Input: dimensioned drawing with shaded views. Units: mm. Origin: part minimum x, y, z. A direction names the side the tool comes from. Coordinates: 2 decimals unless noted, no trailing zeros. Loops run counter-clockwise (first coordinate to the right, second up) from the corner with the lowest first, then second, coordinate; pieces in that order, holes last.
Item 1: Pin query (flat end, axial travel): pin 1 Ø13 at (x, y) = (29, 46.5) entering from -Z; pin 2 Ø12 at (y, z) = (37.5, 120.5) entering from +X. Return the tip coordinate at first contact, or that it passes through.
Item 2: Section query C-C, the plane z = 124. Return the cut outline in (x, y), then the cut area to 3 significant figures.
Item 3: Line query: probe 1 along X at (y, z) = (3, 76.5); probe 2 along Z at (x, y) = (9.5, 31). Output: solid intervals per line, ascending.
Item 4: Section query B-B, the plane x = 30. Return the cut outline in (y, z), then the cut area to 3 significant figures.
Item 5: Reachability of the marked faces 1, 2 and 3 from +Z, -Z, +X, -X, +Y, -Y: full face, straight path, thin tool, end or side. Return the list, or none.
Item 6: Section query A-A, the plane y = 31. Return the cut outline in (x, z), then the cut area to 3 significant figures.
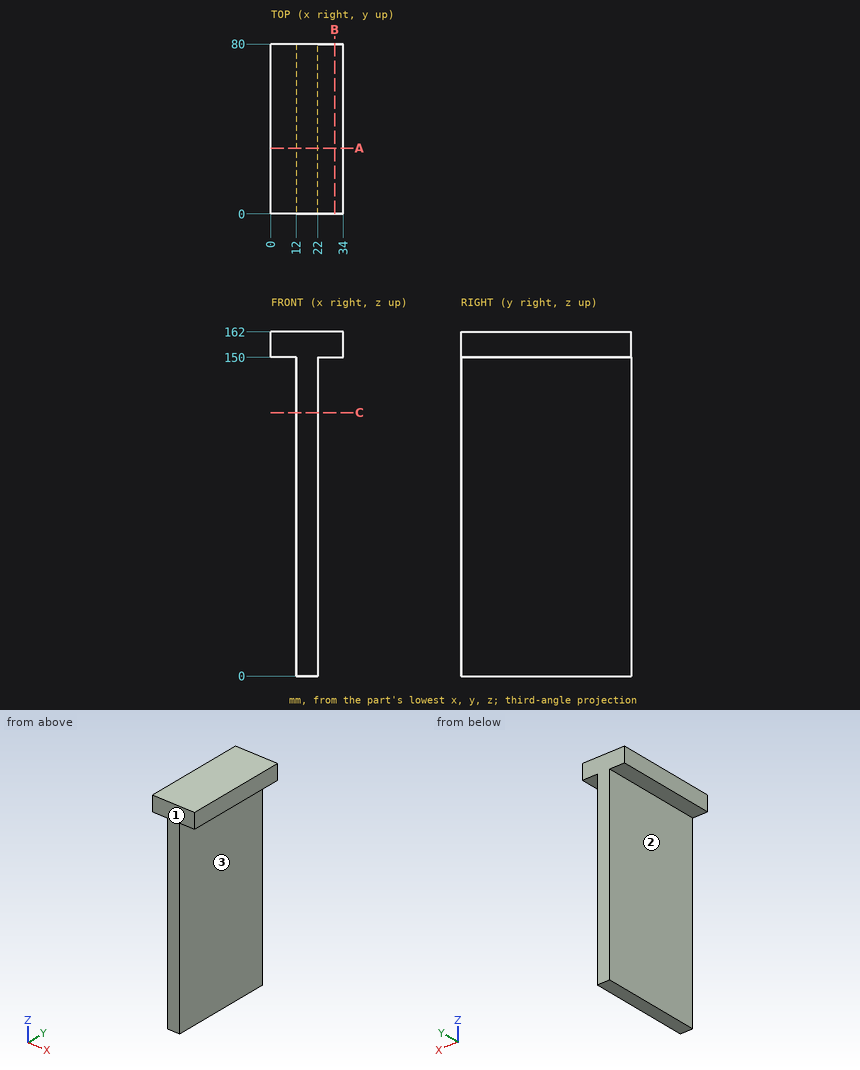
Verdict:
1. pin 1: stops at z = 150
1. pin 2: stops at x = 22
2. outline: (12, 0) - (22, 0) - (22, 80) - (12, 80) - close
2. area: 800 mm2
3. probe 1: x = 12 to 22
3. probe 2: z = 150 to 162
4. outline: (0, 150) - (80, 150) - (80, 162) - (0, 162) - close
4. area: 960 mm2
5. face 1: +Z, -Z, +X, -X, -Y
5. face 2: -Z, -X, +Y, -Y
5. face 3: -Z, +X, +Y, -Y
6. outline: (0, 150) - (12, 150) - (12, 0) - (22, 0) - (22, 150) - (34, 150) - (34, 162) - (0, 162) - close
6. area: 1,910 mm2
